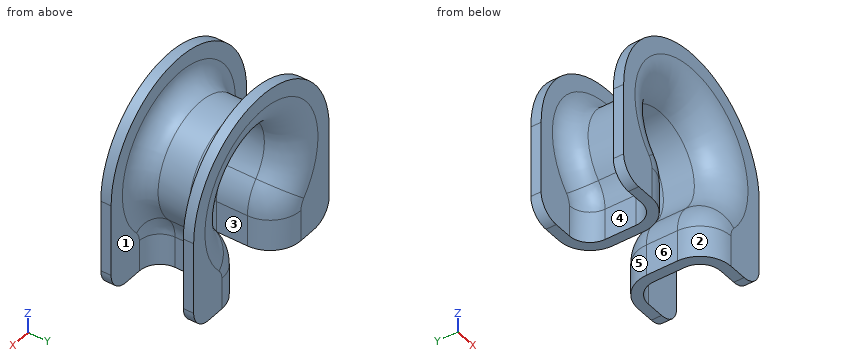
```python
from build123d import *

# Parameters (mm, degrees)
CLIP_BODY_EXTRUDE_18MM_DEPTH = 9
EDGE_FILLETS_R6_R            = 6
SHELL_WALL_2MM_T             = -2


with BuildPart() as part:
    # Clip Profile Sketch → Clip Body Extrude 18mm (new, symmetric)
    with BuildSketch(Plane(origin=(0, 0, 0), x_dir=(1, 0, 0), z_dir=(0, 1, 0))):
        with BuildLine():
            Line((-14, 18), (-4.5, 18))
            Line((-4.5, 18), (-4.5, 11.9058809))
            ThreePointArc((-4.5, 11.9058809), (-5.08127088, 8.723900384), (-6.75, 5.95294045))
            ThreePointArc((-6.75, 5.95294045), (0, -9), (6.75, 5.95294045))
            ThreePointArc((6.75, 5.95294045), (5.08127088, 8.723900384), (4.5, 11.9058809))
            Line((4.5, 11.9058809), (4.5, 18))
            Line((4.5, 18), (14, 18))
            ThreePointArc((14, 18), (16.828427125, 16.828427125), (18, 14))
            Line((18, 14), (18, 0))
            ThreePointArc((18, 0), (0, -18), (-18, 0))
            Line((-18, 0), (-18, 14))
            ThreePointArc((-18, 14), (-16.828427125, 16.828427125), (-14, 18))
        make_face()
    extrude(amount=CLIP_BODY_EXTRUDE_18MM_DEPTH, both=True)

    # Edge Fillets R6
    edge_fillets_r6_edges = [part.edges().sort_by_distance(p)[0] for p in [
        (0, -9, 9),
        (5.08127088, -9, -8.723900384),
        (4.5, -9, -14.95294045),
        (-4.5, -9, -14.95294045),
        (-5.08127088, -9, -8.723900384),
        (4.5, 9, -14.95294045),
        (5.08127088, 9, -8.723900384),
        (0, 9, 9),
        (-5.08127088, 9, -8.723900384),
        (-4.5, 9, -14.95294045),
    ]]
    fillet(edge_fillets_r6_edges, radius=EDGE_FILLETS_R6_R)

    # Shell Wall 2mm
    shell_wall_2mm_openings = [part.faces().sort_by_distance(p)[0] for p in [
        (-9.588709649, 0, -18),
        (-16.828427125, 0, -16.828427125),
        (-18, 0, -7),
        (0, 0, 18),
        (18, 0, -7),
        (16.828427125, 0, -16.828427125),
        (9.588709649, 0, -18),
    ]]
    offset(amount=SHELL_WALL_2MM_T, openings=shell_wall_2mm_openings, kind=Kind.INTERSECTION)


solid = part.part
```
Source: CAD feature listing. Evaluate the final solid. Frame: model axes, mm. Face numbers are marked on the shaded views. A direction names the side the tool comes from. Give positions to 0.01 mm unless a question says otherwise; leave off trailing zeros. Order: outer loops, then holes, each group sorted by start corner. A loop starts at its lowest first (then second) coordinate and runs counter-clockwise, first axis right, second up.
(1) Pull-direction query (Y, two-part tool) for the marked faces 1, 2 and 3; classes: +Y half, -Y half, draft (parallel to the pull), parting line (faces both ways), or undercut.
(2) Material intervals for line 1 along Y through (x, z) = (-9, 15.5); line 2 along X through (y, z) = (-1.7, 0); line 3 along Z through (x, y) = (0, -0.45), sorted ascending.
(3) Section query A-A (x = 0). Return the cut outline in (y, z).
(4) Contact query for flat-ended pins moving along their axis: P1, Ø2, axis at x = -1.5, z = 8.5, coming from the -Y side; P2, Ø5, axis at y = -0.5, z = -16, coming from the +X side; P3, Ø6.5, axis at y = 1.5, z = -14, coming from the +X side. Output: stop coordinate, or through.
(5) Section query C-C (z = -15.5). Return the cut outline in (x, y), plus the area to 3 significant figures.
(6) Section query B-B (y = 2.5). Return the cut outline in (x, z).
(7) Access query for the marked faces 4, 5 and 6. Directions: +Z, -Z, +X, -X, +Y, -Y. A direction counts if a zero-diameter tool reaches every point of the face in a straight line with its end or side. Return the directions, or none.
Outcome:
1. face 1: undercut
1. face 2: -Y half
1. face 3: draft
2. line 1: y = -9 to -7, 7 to 9
2. line 2: x = -11 to -9, 9 to 11
2. line 3: z = 9 to 11
3. outline: (-9, 15) arc R6 ccw to (-3, 9) - (3, 9) arc R6 ccw to (9, 15) - (9, 18) - (7, 18) - (7, 15) arc R4 cw to (3, 11) - (-3, 11) arc R4 cw to (-7, 15) - (-7, 18) - (-9, 18) - close
4. P1: stops at y = -5.68
4. P2: stops at x = 6.5
4. P3: stops at x = 6.9
5. outline: (-17.71, -9) - (-10.5, -9) arc R6 ccw to (-4.5, -3) - (-4.5, 3) arc R6 ccw to (-10.5, 9) - (-17.71, 9) - (-17.71, 7) - (-10.5, 7) arc R4 cw to (-6.5, 3) - (-6.5, -3) arc R4 cw to (-10.5, -7) - (-17.71, -7) - close; (4.5, -3) arc R6 ccw to (10.5, -9) - (17.71, -9) - (17.71, -7) - (10.5, -7) arc R4 cw to (6.5, -3) - (6.5, 3) arc R4 cw to (10.5, 7) - (17.71, 7) - (17.71, 9) - (10.5, 9) arc R6 ccw to (4.5, 3) - close
5. area: 144 mm2
6. outline: (-8.25, -7.28) arc R7 cw to (-6.5, -11.91) - (-6.5, -18) - (-4.5, -18) - (-4.5, -11.91) arc R9 ccw to (-6.75, -5.95) arc R9 cw (long way) to (6.75, -5.95) arc R9 ccw to (4.5, -11.91) - (4.5, -18) - (6.5, -18) - (6.5, -11.91) arc R7 cw to (8.25, -7.28) arc R11 ccw (long way) to start
7. face 4: -Z, -X
7. face 5: -Z, +Y
7. face 6: -Z, +Y, -Y
